Geometry check sheet. Reference: the model listing, model coordinates, mm. A direction names the side the tool comes from. Round coordinates to 2 decimals unless told otherwise and drop trailing zeros. Loops run counter-clockwise (first coordinate to the right, second up) from the corner with the lowest first, then second, coordinate; pieces in that order, holes last. Notation, with made-up numbers: (12.25, 34) -> (68.25, 34) arc R20 cw to (68.25, 64) -> close; hole circle Ø4 at (73.5, 46). An arc over 180 degrees is marked (long way). Use one line per item in the form item = value.
from build123d import *

# Parameters (mm, degrees)
LPATTERN1_COUNT          = 2
LPATTERN1_PITCH          = 180
SKETCH3_R                = 22.5
BOSS_EXTRUDE2_DEPTH      = 135
SKETCH4_R                = 30.412434653
SKETCH4_R_2              = 16
CUT_EXTRUDE1_DEPTH       = 2
SKETCH5_R                = 8
BOSS_EXTRUDE3_DEPTH      = 47
LPATTERN2_COUNT          = 2
LPATTERN2_PITCH          = 180
BOSS_EXTRUDE4_DEPTH      = 20
BOSS_EXTRUDE4_DEPTH_BACK = 45
SKETCH6_W                = 131
SKETCH6_H                = 225
SKETCH7_R                = 65
BOSS_EXTRUDE5_DEPTH      = 20
CUT_EXTRUDE2_DEPTH       = 342.400058582
CUT_EXTRUDE2_DEPTH_BACK  = 342.400058582
SKETCH8_R                = 45


with BuildPart() as part:
    # Sketch2 → Revolve1 (revolve)
    with BuildSketch(Plane(origin=(0, 0, 0), x_dir=(1, 0, 0), z_dir=(0, 1, 0)), mode=Mode.PRIVATE) as revolve1_sk:
        Polygon((0, 0), (0, 35), (5.386751346, 35), (19.820508076, 10), (25.179491924, 10), (39.613248654, 35), (45, 35), (45, 0), align=None)
    revolve(revolve1_sk.sketch.rotate(Axis((10.892128266, 0, 8), (1, 0, 0)), 180), axis=Axis((10.892128266, 0, 8), (1, 0, 0)))


with BuildPart() as lpattern1_1:
    # LPattern1: pattern copy
    add(part.part.moved(Location(Vector(1, 0, 0) * (1 * LPATTERN1_PITCH))))


with BuildPart() as part_1:
    add(part.part)

    add(lpattern1_1.part)  # Boss-Extrude2 merges LPattern1_1
    # Sketch3 → Boss-Extrude2 (add)
    with BuildSketch(Plane(origin=(45, 0, 0), x_dir=(0, 0, -1), z_dir=(1, 0, 0))):
        with Locations(Location((-8, 0, 0), (0, 0, 180))):
            Circle(SKETCH3_R)
    extrude(amount=BOSS_EXTRUDE2_DEPTH)

    # Sketch4 → Cut-Extrude1 (cut)
    with BuildSketch(Plane(origin=(45, 0, 0), x_dir=(0, 0, -1), z_dir=(1, 0, 0))):
        with Locations((-8, 0)):
            Circle(SKETCH4_R)
        with Locations((-8, 0)):
            Circle(SKETCH4_R_2, mode=Mode.SUBTRACT)
    cut_extrude1 = extrude(amount=CUT_EXTRUDE1_DEPTH, mode=Mode.SUBTRACT)

    # Mirror1: Cut-Extrude1 across plane
    add(cut_extrude1.mirror(Plane.ZY.offset(-112.5)), mode=Mode.SUBTRACT)

    # Sketch5 → Boss-Extrude3 (add)
    with BuildSketch(Plane(origin=(180, 0, 0), x_dir=(0, 0, -1), z_dir=(1, 0, 0))):
        with Locations(Location((-8, 0, 0), (0, 0, 180))):
            Circle(SKETCH5_R)
    boss_extrude3 = extrude(amount=BOSS_EXTRUDE3_DEPTH)

    # Mirror2: Boss-Extrude3 across plane
    add(boss_extrude3.mirror(Plane.ZY.offset(-112.5)))


with BuildPart() as lpattern2_1:
    # LPattern2: pattern copy
    add(part_1.part.moved(Location(Vector(0, 0, 1) * (1 * LPATTERN2_PITCH))))


with BuildPart() as part_2:
    add(part_1.part)

    add(lpattern2_1.part)  # Boss-Extrude4 merges LPattern2_1
    # Sketch6 → Boss-Extrude4 (add, two sides: drawn at the far end of the back side and taken through both)
    with BuildSketch(Plane(origin=(0, 0, 0), x_dir=(1, 0, 0), z_dir=(0, 1, 0)).offset(-BOSS_EXTRUDE4_DEPTH_BACK)):
        with Locations((112.5, -98)):
            Rectangle(SKETCH6_W, SKETCH6_H)
    extrude(amount=BOSS_EXTRUDE4_DEPTH + BOSS_EXTRUDE4_DEPTH_BACK)

    # Sketch7 → Boss-Extrude5 (add)
    with BuildSketch(Plane.XZ.offset(45)):
        with Locations(Location((112.5, 97.931490015, 0), (0, 0, 270))):
            Circle(SKETCH7_R)
    extrude(amount=BOSS_EXTRUDE5_DEPTH)

    # Sketch8 → Cut-Extrude2 (cut, two sides: drawn at the far end of the back side and taken through both)
    with BuildSketch(Plane.XZ.offset(65).offset(-CUT_EXTRUDE2_DEPTH_BACK)):
        with Locations(Location((112.5, 97.931490015, 0), (0, 0, 270))):
            Circle(SKETCH8_R)
    extrude(amount=CUT_EXTRUDE2_DEPTH + CUT_EXTRUDE2_DEPTH_BACK, mode=Mode.SUBTRACT)


solid = part_2.part
1. Section check A-A (x = 112.5). Record the boundary of the cut face in (y, z), then the cut area to 3 significant figures.
Return value:
outline = (-65, 32.93) -> (-45, 32.93) -> (-45, -14.5) -> (20, -14.5) -> (20, -2.31) arc R22.5 ccw to (20, 18.31) -> (20, 52.93) -> (-65, 52.93) -> close; (-65, 142.93) -> (20, 142.93) -> (20, 177.69) arc R22.5 ccw to (20, 198.31) -> (20, 210.5) -> (-45, 210.5) -> (-45, 162.93) -> (-65, 162.93) -> close
area = 9,640 mm2
2. Section check C-C (y = -53). Record the boundary of the cut face in (x, z), then the cut area to 3 significant figures.
Return value:
outline = circle Ø130 at (112.5, 97.93); hole circle Ø90 at (112.5, 97.93)
area = 6,910 mm2
3. Tool access check on faces 5 (the cylindrical face through (179.014, 0.703, 203.985)), 6 (the flat face through (227, 0, 188)), 7 (the cylindrical face through (-1, 0, 180)), 8 (the cylindrical face through (226, 0, 180)), 9 (the flat face through (112, 20, -8)). Record the directions out of +Z, -Z, +X, -X, +Y, -Y that give a thin tool (end or side, any length) a straight path to the whole face; none if there is none.
Return value:
face_5 = none
face_6 = +Z, -Z, +X, +Y, -Y
face_7 = -X
face_8 = +X
face_9 = -Z, +Y
4. Gauge pin test, flat ends, axial feed: pin 1 (10 mm diameter, centred on y = 19.5, z = 140, fed in from -X); pin 2 (6 mm diameter, centred on x = 114.5, z = 202, fed in from +Y); pin 3 (10 mm diameter, centred on x = 139, y = -33, fed in from -Z). Record the tip position at first contact, or that the pin passes through.
Return value:
pin_1 = 47
pin_2 = 20
pin_3 = -14.5
5. Mould release check, pull along Z, two halves, no side actions. Record for faces 1 (the flat face through (227, 0, 8)), 2 (the conical face through (19.12, -19.05, 5.5)), 3 (the cylindrical face through (132.02, -54.86, 35.93)), 4 (the flat face through (112, -13, -14.5)): released by +Z, released by -Z, zero draft, split by the parting line, or undercut.
Return value:
face_1 = zero draft
face_2 = undercut
face_3 = split by the parting line
face_4 = released by -Z
6. Section check D-D (y = -28.5). Count the separate pieces of the cut face and the enclosed holes in it, then the cut area to 3 significant figures.
Return value:
separate_pieces = 9
enclosed_holes = 1
area = 28,600 mm2
7. Material ranges on line 1 along Z through (x, y) = (112.5, -18); line 2 along X through (y, z) = (8, 99.5); line 3 along X through (y, z) = (34, 2), recorded low to high.
Return value:
line_1 = -14.5 to 52.93, 142.93 to 210.5
line_2 = 47 to 67.53, 157.47 to 178
line_3 = 0 to 10.28, 34.72 to 45, 180 to 190.28, 214.72 to 225
8. Section check B-B (z = 104). Record the boundary of the cut face in (x, y), then the cut area to 3 significant figures.
Return value:
outline = (47, -45) -> (47.78, -45) -> (47.78, -65) -> (67.91, -65) -> (67.91, 20) -> (47, 20) -> close; (157.09, -65) -> (177.22, -65) -> (177.22, -45) -> (178, -45) -> (178, 20) -> (157.09, 20) -> close
area = 3,520 mm2
